Read the model definition and answer for the solid it produces. Units are mm, in the model's axes. Round coordinates to 2 decimals unless told otherwise and drop trailing zeros. Order: outer loops, then holes, each group sorted by start corner. A loop starts at its lowest first (then second) coordinate and runs counter-clockwise, first axis right, second up.
from build123d import *

# Parameters (mm, degrees)
SKETCH1_R               = 7.5
SKETCH1_R_2             = 6
BOSS_EXTRUDE1_DEPTH     = 700
CUT_EXTRUDE1_DEPTH      = 701.080352531
CUT_EXTRUDE1_DEPTH_BACK = 701.080352531
SKETCH2_R               = 3


with BuildPart() as part:
    # Sketch1 → Boss-Extrude1 (new body)
    with BuildSketch(Plane.XY):
        Circle(SKETCH1_R)
        Circle(SKETCH1_R_2, mode=Mode.SUBTRACT)
    extrude(amount=BOSS_EXTRUDE1_DEPTH)

    # Sketch2 → Cut-Extrude1 (cut, two sides: drawn at the far end of the back side and taken through both)
    with BuildSketch(Plane(origin=(0, 0, 0), x_dir=(1, 0, 0), z_dir=(0, 1, 0)).offset(-CUT_EXTRUDE1_DEPTH_BACK)):
        with Locations(Location((0, -10, 0), (0, 0, 270))):
            Circle(SKETCH2_R)
        with Locations(Location((0, -690, 0), (0, 0, 270))):
            Circle(SKETCH2_R)
    extrude(amount=CUT_EXTRUDE1_DEPTH + CUT_EXTRUDE1_DEPTH_BACK, mode=Mode.SUBTRACT)


solid = part.part
Q1. Straight lines are drawn through the part: probe 1 along Z at (x, y) = (-0.75, -6.5); probe 2 along Z at (x, y) = (1.5, 7); probe 3 along Y at (x, z) = (0, 352.5). For each, find the intervals that lie inside material, in ascending order.
Outcome:
probe 1: z = 0 to 7.1, 12.9 to 687.1, 692.9 to 700
probe 2: z = 0 to 7.4, 12.6 to 687.4, 692.6 to 700
probe 3: y = -7.5 to -6, 6 to 7.5
Q2. A cutting plane is placed at B-B, the plane x = 0. Give the vertices of the cut face in (y, z).
Outcome:
outline: (-7.5, 0) - (-6, 0) - (-6, 7) - (-7.5, 7) - close; (-7.5, 13) - (-6, 13) - (-6, 687) - (-7.5, 687) - close; (-7.5, 693) - (-6, 693) - (-6, 700) - (-7.5, 700) - close; (6, 0) - (7.5, 0) - (7.5, 7) - (6, 7) - close; (6, 13) - (7.5, 13) - (7.5, 687) - (6, 687) - close; (6, 693) - (7.5, 693) - (7.5, 700) - (6, 700) - close
Q3. A cutting plane is placed at A-A, the plane y = 0. Give the vertices of the cut face in (x, z).
Outcome:
outline: (-7.5, 0) - (-6, 0) - (-6, 700) - (-7.5, 700) - close; (6, 0) - (7.5, 0) - (7.5, 700) - (6, 700) - close
Q4. Flat-ended cylindrical pins translate along their axes: pin 1 (5 mm diameter, centred on x = 0, z = 690, fed in from -Y); pin 2 (1 mm diameter, centred on y = 4.5, z = 87.5, fed in from +X); pin 3 (1.5 mm diameter, centred on y = 5, z = 150, fed in from +X); pin 4 (6 mm diameter, centred on x = 5.5, z = 244.5, fed in from -Y). Find the tip coordinate at first contact, or state that the pin passes through.
Outcome:
pin 1: passes through
pin 2: stops at x = 6.34
pin 3: stops at x = 6.18
pin 4: stops at y = -7.07
Q5. For a pull along Y with two mould halves and no side action, classify faces 1 (the face through (2, 6, 700)), 2 (the face through (-6, 0, 345)), 3 (the face through (-7.493, 0.33, 345.1)) as released by +Y, released by -Y, zero draft, split by the parting line, or undercut.
Outcome:
face 1: zero draft
face 2: undercut
face 3: split by the parting line
Q6. A cutting plane is placed at C-C, the plane z = 255. Give the vertices of the cut face in (x, y).
Outcome:
outline: circle Ø15 at (0, 0); hole circle Ø12 at (0, 0)
